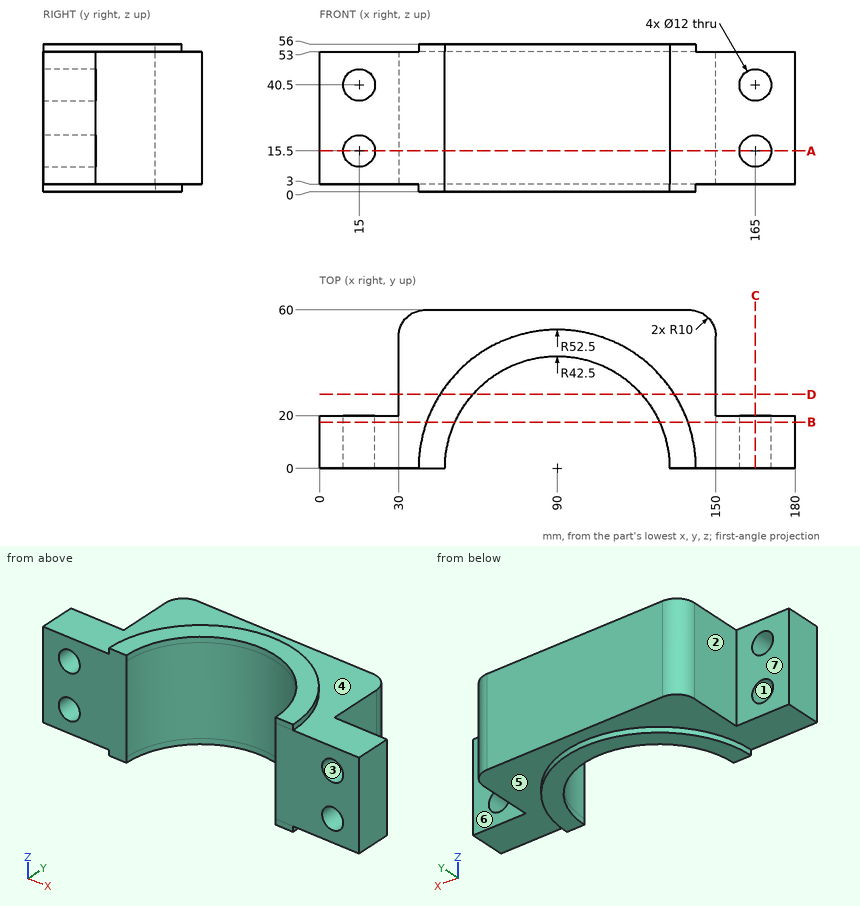
Part print with two shaded views. Sizes in mm from the minimum x, y, z corner. A direction names the side the tool comes from. Round coordinates to 2 decimals unless told otherwise and drop trailing zeros. Loops run counter-clockwise (first coordinate to the right, second up) from the corner with the lowest first, then second, coordinate; pieces in that order, holes last. Notation, with made-up numbers: M -18,-6 L 31,-6 A18 cw 31,12 Z; hole C 75.5,70.25 d9. An arc over 180 degrees is marked long. Return JSON: item names as keys, results as strings. Group by question number.
(1) Saw through at C-C, the plane x = 165. List the corners of the cut face in (y, z), and give its area (3 significant figures).
(2) Tool access for the marked faces 5, 6 and 7: list every direction of +Z, -Z, +X, -X, +Y, -Y with a clear straight run to the whole face (end or side of a thin tool).
(3) Wall check: probe 1 along X at (y, z) = (14.25, 15.5); probe 2 along X at (y, z) = (10, 15.5); probe 3 along X at (y, z) = (29.5, 27.5). Give the ranges that are in metal, low to high. Write a range as [from, to].
(4) Saw through at D-D, the plane y = 28. List the corners of the cut face in (x, z), and give its area (3 significant figures).
(5) Saw through at B-B, the plane y = 17.5. List the corners of the cut face in (x, z).
(6) Drop flat-ended pins along their axis: P1, Ø5, axis at y = 45, z = 6.5, coming from the -X side; P2, Ø2, axis at x = 58.5, y = 49.5, coming from the -Z side; P3, Ø24, axis at x = 165.5, z = 18.5, coming from the +Y side; P4, Ø18, axis at x = 106, y = 22.5, coming from the -Z side. Give the stop position or say it passes through.
(7) Mould opens along Z. For the marked faces 1, 2, 3 and 4 say: +Z half, -Z half, draft (parallel to the pull), parting line (faces both ways), or undercut.
(8) Saw through at A-A, the plane z = 15.5. List the corners of the cut face in (x, y).
Answer list:
{
 "1": {"outline": "M 0,3 L 20,3 L 20,9.5 L 0,9.5 Z; M 0,21.5 L 20,21.5 L 20,34.5 L 0,34.5 Z; M 0,46.5 L 20,46.5 L 20,53 L 0,53 Z", "area": "520 mm2"},
 "2": {"face 5": "-Z, +Y", "face 6": "+Z, -Z, +X, +Y", "face 7": "+Z, -Z, -X, +Y"},
 "3": {"probe 1": "[0, 9], [21, 49.96], [130.04, 159], [171, 180]", "probe 2": "[0, 9], [21, 48.69], [131.31, 159], [171, 180]", "probe 3": "[30, 59.41], [120.59, 150]"},
 "4": {"outline": "M 30,3 L 45.59,3 L 45.59,0 L 58.03,0 L 58.03,56 L 45.59,56 L 45.59,53 L 30,53 Z; M 121.97,0 L 134.41,0 L 134.41,3 L 150,3 L 150,53 L 134.41,53 L 134.41,56 L 121.97,56 Z", "area": "2,950 mm2"},
 "5": {"outline": "M 0,3 L 40.5,3 L 40.5,0 L 51.27,0 L 51.27,56 L 40.5,56 L 40.5,53 L 0,53 Z; M 128.73,0 L 139.5,0 L 139.5,3 L 180,3 L 180,53 L 139.5,53 L 139.5,56 L 128.73,56 Z; hole C 15,15.5 d12; hole C 15,40.5 d12; hole C 165,15.5 d12; hole C 165,40.5 d12"},
 "6": {"P1": "x = 30", "P2": "z = 3", "P3": "y = 20", "P4": "through"},
 "7": {"face 1": "undercut", "face 2": "draft", "face 3": "undercut", "face 4": "+Z half"},
 "8": {"outline": "M 0,0 L 9,0 L 9,20 L 0,20 Z; M 21,0 L 47.5,0 A42.5 cw 132.5,0 L 159,0 L 159,20 L 150,20 L 150,50 A10 ccw 140,60 L 40,60 A10 ccw 30,50 L 30,20 L 21,20 Z; M 171,0 L 180,0 L 180,20 L 171,20 Z"}
}
